```python
from build123d import *

# Parameters (mm, degrees)
SKETCH_1_R          = 35
EXTRUDE_1_DEPTH     = 45
SKETCH_5_R          = 37.5
EXTRUDE_2_DEPTH     = 18
CHAMFER_1_SIZE      = 5
HOLE_WIZARD_M20_1_D = 17.5
FILLET_1_R          = 0.5


with BuildPart() as part:
    # 草图1 → 凸台-拉伸1 (new body)
    with BuildSketch(Plane.XY):
        with Locations(Location((0, 0, 0), (0, 0, 180))):
            Circle(SKETCH_1_R)
    extrude(amount=EXTRUDE_1_DEPTH)

    # 草图5 → 凸台-拉伸2 (add)
    with BuildSketch(Plane(origin=(0, 0, 0), x_dir=(-1, 0, 0), z_dir=(0, 0, -1))):
        Circle(SKETCH_5_R)
    extrude(amount=EXTRUDE_2_DEPTH)

    # 倒角1
    chamfer_1_edges = [part.edges().sort_by_distance(p)[0] for p in [
        (35, 0, 45),
        (37.5, 0, -18),
    ]]
    chamfer(chamfer_1_edges, length=CHAMFER_1_SIZE)

    # M20 螺纹孔1 (through all)
    with Locations(Plane(origin=(-0.093425474, -0.140138211, 45), x_dir=(1, 0, 0), z_dir=(0, 0, 1))):
        with Locations((0, 0)):
            Hole(HOLE_WIZARD_M20_1_D / 2)

    # 圆角1
    fillet_1_edges = [part.edges().sort_by_distance(p)[0] for p in [
        (35, 0, 0),
    ]]
    fillet(fillet_1_edges, radius=FILLET_1_R)


solid = part.part
```
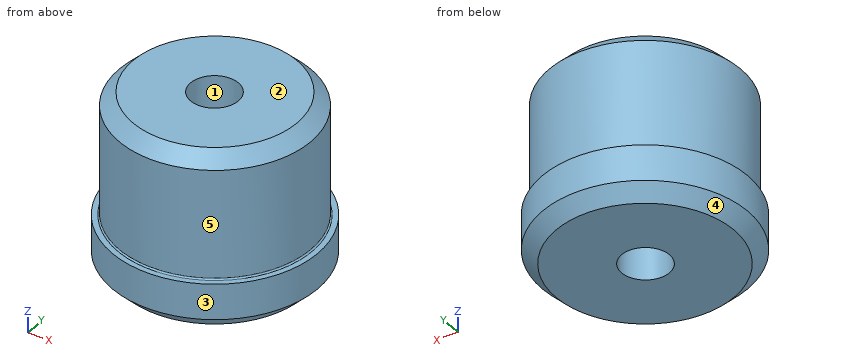
Can you work these out from the model? Positions are in its coordinate system, mm. Face numbers are marked on the shaded views. A direction names the side the tool comes from. Coordinates: 2 decimals unless noted, no trailing zeros. Loops run counter-clockwise (first coordinate to the right, second up) from the corner with the lowest first, then second, coordinate; pieces in that order, holes last.
Item 1: If we mould it in two halves opening along Y, with no side actions, what happens to the marked faces 1, 2 and 3? For each: released by +Y, released by -Y, zero draft, split by the parting line, or undercut.
Answers below:
face 1: undercut
face 2: zero draft
face 3: split by the parting line
Item 2: Which directions (+Z, -Z, +X, -X, +Y, -Y) give clear straight access to the entire face, cutting with the end or side of a thin tool? Please do the marked faces 4 and 5.
Answers below:
face 4: -Z
face 5: +Z
Item 3: Suppose I cut it at C-C (z = -9.5). Please give me the cut outline in (x, y), then the cut area to 3 significant figures.
Answers below:
outline: circle Ø75 at (0, 0); hole circle Ø17.5 at (-0.09, -0.14)
area: 4,180 mm2
Item 4: Suppose I cut it at B-B (z = 37.5). Please give me the cut outline in (x, y).
Answers below:
outline: circle Ø70 at (0, 0); hole circle Ø17.5 at (-0.09, -0.14)
Item 5: Please list where these lines run through material, in increasing order: L1, parallel to X at y = -3, z = 39; L2, parallel to Y at x = 13, z = 36; L3, parallel to Y at x = -22.5, z = -12.
Answers below:
L1: x = -34.87 to -8.36, 8.18 to 34.87
L2: y = -32.5 to 32.5
L3: y = -30 to 30
Item 6: Suppose I cut it at A-A (x = 0). Please give me the cut outline in (y, z).
Answers below:
outline: (-37.5, -13) - (-32.5, -18) - (-8.89, -18) - (-8.89, 45) - (-30, 45) - (-35, 40) - (-35, 0.5) arc R0.5 cw to (-35.5, 0) - (-37.5, 0) - close; (8.61, -18) - (32.5, -18) - (37.5, -13) - (37.5, 0) - (35.5, 0) arc R0.5 cw to (35, 0.5) - (35, 40) - (30, 45) - (8.61, 45) - close
Item 7: I'm going to push flat-ended pins straight in: pin 1 (4 mm diameter, centred on y = 6, z = 19, fed in from +X); pin 2 (5 mm diameter, centred on x = 22.5, y = 26.5, fed in from +Z); pin 3 (1 mm diameter, centred on x = -3, z = 27.5, fed in from +Y). Where does each tip first touch, or does it pass through?
Answers below:
pin 1: stops at x = 34.77
pin 2: stops at z = 42.74
pin 3: stops at y = 34.91
